Could you check a few things on this model? Use its own coordinates, in mm. A direction names the side the tool comes from. Coordinates: 2 decimals unless noted, no trailing zeros. Write each loop counter-clockwise with the first axis right and the second up, starting at its lowest first coordinate (ties: lowest second). Pieces come first, ordered by that corner, then holes. Notation, with made-up numbers: M 4,29.5 L 18,29.5 A27 cw 18,57.5 Z; hole C 15.5,51.5 d8. An arc over 180 degrees is marked long. Answer as CSV lines item,"result". Start each with the question number.
Item 1: Suppose I cut it at A-A, the plane x = 30. Write out the boundary of the cut face in (y, z), and give its area (3 significant figures).
Item 2: Suppose I cut it at D-D, the plane x = 65. Write out the boundary of the cut face in (y, z).
Item 3: On a 3-axis mill with a long thin cutter (end or side, diameter ignored), from which of +Z, -Z, +X, -X, +Y, -Y can I reach the whole of each face in a straight line? I mean faces 1 (the flat face through (54, 5.5, -65)), 2 (the cylindrical face through (12.4, 6, -6)), 3 (the flat face through (5, 3, -70)). Say none if no direction works.
Item 4: Suppose I cut it at C-C, the plane z = -76.5. Write out the boundary of the cut face in (x, y).
Item 5: If I drill on line 1 along X through (y, z) = (5.5, -17.5); line 2 along X through (y, z) = (2.25, -31); line 3 along Z through (x, y) = (56, 6.25), over which ranges is the centre line in solid material (lowest first)? Write a range as [from, to].
Item 6: Suppose I cut it at B-B, the plane z = -66. State how many separate pieces and enclosed holes the cut face has, and give its area (4 significant figures).
Item 7: We'd pull the mould along Z, two halves only. Please class faces 4 (the cylindrical face through (97.6, 6, -58)), 5 (the flat face through (105, 3, -70)), 6 (the flat face through (54, 9, -80)): +Z half, -Z half, draft (parallel to the pull), parting line (faces both ways), or undercut.
Item 8: I'm going to push flat-ended pins straight in: P1, Ø3, axis at x = 56.5, z = -66.5, coming from the +Y side; P2, Ø3.5, axis at x = 4, y = 2, coming from the -Z side. Where does each tip first touch, or does it pass through?
```python
from build123d import *

# Parameters (mm, degrees)
SKETCH1_W             = 110
SKETCH1_H             = 90
BOSS_EXTRUDE1_DEPTH   = 9
SKETCH2_W             = 110
SKETCH2_H             = 8
BOSS_EXTRUDE2_DEPTH   = 1.5
SKETCH5_W             = 20
SKETCH5_H             = 20
BOSS_EXTRUDE3_DEPTH   = 9
CUT_EXTRUDE1_DEPTH    = 156.823618235
CUT_EXTRUDE2_DEPTH    = 6
SKETCH6_W             = 10
SKETCH6_H             = 40
CUT_EXTRUDE3_DEPTH    = 156.823618235
SKETCH8_W             = 110
SKETCH8_H             = 9
CUT_EXTRUDE5_DEPTH    = 5
M3_TAPPED_HOLE1_D     = 2.5
MOVE_FACE1_BY         = 20
MOVE_FACE1_2_BY       = 20
F_3_0MM_DOWEL_HOLE1_D = 3
CHAMFER1_SIZE         = 0.5
CHAMFER3_SIZE         = 0.5
CHAMFER4_SIZE         = 0.5


with BuildPart() as part:
    # Sketch1 → Boss-Extrude1 (new body)
    with BuildSketch(Plane(origin=(0, 0, 0), x_dir=(1, 0, 0), z_dir=(0, 1, 0))):
        with Locations((55, 45)):
            Rectangle(SKETCH1_W, SKETCH1_H)
    extrude(amount=BOSS_EXTRUDE1_DEPTH)

    # Sketch2 → Boss-Extrude2 (add)
    with BuildSketch(Plane(origin=(0, 9, 0), x_dir=(1, 0, 0), z_dir=(0, 1, 0))):
        with Locations((55, 66)):
            Rectangle(SKETCH2_W, SKETCH2_H)
    extrude(amount=BOSS_EXTRUDE2_DEPTH)

    # Sketch5 → Boss-Extrude3 (add)
    with BuildSketch(Plane.XZ):
        with Locations((10, -100)):
            Rectangle(SKETCH5_W, SKETCH5_H)
        with Locations((100, -100)):
            Rectangle(SKETCH5_W, SKETCH5_H)
    extrude(amount=-BOSS_EXTRUDE3_DEPTH)

    # Sketch3 → Cut-Extrude1 (cut, through all)
    with BuildSketch(Plane(origin=(0, 9, 0), x_dir=(1, 0, 0), z_dir=(0, 1, 0))):
        with BuildLine():
            Line((15.5, 52), (15.5, 12))
            ThreePointArc((15.5, 12), (12.5, 9), (9.5, 12))
            Line((9.5, 12), (9.5, 52))
            ThreePointArc((9.5, 52), (12.5, 55), (15.5, 52))
        make_face()
        with BuildLine():
            Line((94.5, 52), (94.5, 12))
            ThreePointArc((94.5, 12), (97.5, 9), (100.5, 12))
            Line((100.5, 12), (100.5, 52))
            ThreePointArc((100.5, 52), (97.5, 55), (94.5, 52))
        make_face()
    extrude(amount=-CUT_EXTRUDE1_DEPTH, mode=Mode.SUBTRACT)

    # Sketch4 → Cut-Extrude2 (cut)
    with BuildSketch(Plane(origin=(0, 9, 0), x_dir=(1, 0, 0), z_dir=(0, 1, 0))):
        with BuildLine():
            Line((6.5, 52), (6.5, 12))
            ThreePointArc((6.5, 12), (12.5, 6), (18.5, 12))
            Line((18.5, 12), (18.5, 52))
            ThreePointArc((18.5, 52), (12.5, 58), (6.5, 52))
        make_face()
        with BuildLine():
            Line((103.5, 12), (103.5, 52))
            ThreePointArc((103.5, 52), (97.5, 58), (91.5, 52))
            Line((91.5, 52), (91.5, 12))
            ThreePointArc((91.5, 12), (97.5, 6), (103.5, 12))
        make_face()
    extrude(amount=-CUT_EXTRUDE2_DEPTH, mode=Mode.SUBTRACT)

    # Sketch6 → Cut-Extrude3 (cut, through all)
    with BuildSketch(Plane(origin=(0, 9, 0), x_dir=(1, 0, 0), z_dir=(0, 1, 0))):
        with Locations((5, 90)):
            Rectangle(SKETCH6_W, SKETCH6_H)
        with Locations((105, 90)):
            Rectangle(SKETCH6_W, SKETCH6_H)
    extrude(amount=-CUT_EXTRUDE3_DEPTH, mode=Mode.SUBTRACT)

    # Sketch8 → Cut-Extrude5 (cut)
    with BuildSketch(Plane(origin=(0, 10.5, 0), x_dir=(1, 0, 0), z_dir=(0, 1, 0))):
        with Locations((55, 65.5)):
            Rectangle(SKETCH8_W, SKETCH8_H)
    extrude(amount=-CUT_EXTRUDE5_DEPTH, mode=Mode.SUBTRACT)

    # M3 Tapped Hole1 (through all)
    with Locations(Plane(origin=(0, 5.5, 0), x_dir=(1, 0, 0), z_dir=(0, 1, 0))):
        with Locations((10, 66), (100, 66), (20, 66), (90, 66)):
            Hole(M3_TAPPED_HOLE1_D / 2)

    # Move Face1: a face moved inward by 20.0
    extrude(part.faces().sort_by_distance((95, 4.5, -110))[0], amount=MOVE_FACE1_BY, dir=(0, 0, 1), mode=Mode.SUBTRACT)

    # Move Face1 2: a face moved inward by 20.0
    extrude(part.faces().sort_by_distance((15, 4.5, -110))[0], amount=MOVE_FACE1_2_BY, dir=(0, 0, 1), mode=Mode.SUBTRACT)

    # Ø3.0mm dowel hole1 (through all)
    with Locations(Plane(origin=(0, 5.5, 0), x_dir=(1, 0, 0), z_dir=(0, 1, 0))):
        with Locations((30, 66), (80, 66)):
            Hole(F_3_0MM_DOWEL_HOLE1_D / 2)

    # Chamfer1
    chamfer1_edges = [part.edges().sort_by_distance(p)[0] for p in [
        (0, 0, -35),
        (110, 9, -30.5),
        (10, 4.5, -90),
        (100, 4.5, -90),
        (110, 2.75, -70),
        (0, 2.75, -70),
        (0, 9, -30.5),
        (110, 7.25, -61),
        (0, 7.25, -61),
        (0, 5.5, -65.5),
        (110, 5.5, -65.5),
        (55, 9, -90),
        (55, 0, -90),
        (110, 0, -35),
        (55, 0, 0),
        (110, 4.5, 0),
        (0, 4.5, 0),
        (55, 9, 0),
    ]]
    chamfer(chamfer1_edges, length=CHAMFER1_SIZE)

    # Chamfer3
    chamfer3_edges = [part.edges().sort_by_distance(p)[0] for p in [
        (55, 9, -70),
        (10, 0, -79.75),
        (10, 9, -79.75),
        (104.75, 0, -70),
        (5.25, 5.5, -70),
        (100, 0, -79.75),
        (5.25, 0, -70),
        (100, 9, -79.75),
        (104.75, 5.5, -70),
        (55, 9, -61),
    ]]
    chamfer(chamfer3_edges, length=CHAMFER3_SIZE)

    # Chamfer4
    chamfer4_edges = [part.edges().sort_by_distance(p)[0] for p in [
        (10, 7, -70),
        (100, 7, -70),
    ]]
    chamfer(chamfer4_edges, length=CHAMFER4_SIZE)


solid = part.part
```
Ans:
1,outline,"M 0,-89.5 L 0.5,-90 L 8.5,-90 L 9,-89.5 L 9,-70.5 L 8.5,-70 L 5.5,-70 L 5.5,-67.5 L 0,-67.5 Z; M 0,-64.5 L 5.5,-64.5 L 5.5,-61 L 8.5,-61 L 9,-60.5 L 9,-0.5 L 8.5,0 L 0.5,0 L 0,-0.5 Z"
1,area,"761 mm^2"
2,outline,"M 0,-89.5 L 0.5,-90 L 8.5,-90 L 9,-89.5 L 9,-70.5 L 8.5,-70 L 5.5,-70 L 5.5,-61 L 8.5,-61 L 9,-60.5 L 9,-0.5 L 8.5,0 L 0.5,0 L 0,-0.5 Z"
3,face 1,"+X, -X, +Y"
3,face 2,"+Y"
3,face 3,"-Z, -X, +Y, -Y"
4,outline,"M 10,0.5 L 10.5,0 L 99.5,0 L 100,0.5 L 100,8.5 L 99.5,9 L 10.5,9 L 10,8.5 Z"
5,line 1,"x = [0, 6.5], [18.5, 91.5], [103.5, 110]"
5,line 2,"x = [0, 9.5], [15.5, 94.5], [100.5, 110]"
5,line 3,"z = [-90, -70], [-61, 0]"
6,separate pieces,"7"
6,enclosed holes,"0"
6,area,"516.5 mm^2"
7,face 4,"undercut"
7,face 5,"-Z half"
7,face 6,"draft"
8,P1,"stops at y = 5.5"
8,P2,"stops at z = -70"
